```python
from build123d import *

# Parameters (mm, degrees)
LINK_PROFILE_SKETCH_R = 2.5
LINK_BAR_4MM_DEPTH    = 2


with BuildPart() as part:
    # Link Profile Sketch → Link Bar 4mm (new, symmetric)
    with BuildSketch(Plane.XY):
        with BuildLine():
            Line((-45, 5), (45, 5))
            ThreePointArc((45, 5), (50, 0), (45, -5))
            Line((45, -5), (-45, -5))
            ThreePointArc((-45, -5), (-50, 0), (-45, 5))
        make_face()
        with Locations((-45, 0)):
            Circle(LINK_PROFILE_SKETCH_R, mode=Mode.SUBTRACT)
        with Locations((45, 0)):
            Circle(LINK_PROFILE_SKETCH_R, mode=Mode.SUBTRACT)
    extrude(amount=LINK_BAR_4MM_DEPTH, both=True)


solid = part.part
```
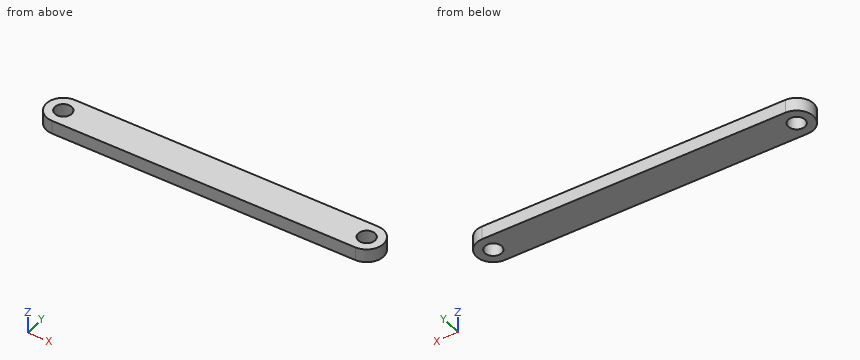
Model file for the job. Use its own axes, mm. Coordinates: 2 decimals unless noted, no trailing zeros. Order: outer loops, then holes, each group sorted by start corner. A loop starts at its lowest first (then second) coordinate and runs counter-clockwise, first axis right, second up. Notation, with made-up numbers: (52, 65.25) -> (107, 65.25) arc R26 cw to (107, 102.25) -> close; hole circle Ø6 at (5, -8.5). An arc over 180 degrees is marked (long way). Answer as a JSON object with one key per item and string values. Group by question number.
1) Drill centre lines: L1, parallel to Y at x = -45, z = 0.75; L2, parallel to X at y = 1, z = 0.4; L3, parallel to X at y = 0.5, z = -0.45. Where is each one in solid material? Low to high.
2) Cut at C-C, the plane y = 4. Write the cut outline in (x, z), then the cut area to 3 significant figures.
3) Cut at D-D, the plane y = -3.75. Write the cut outline in (x, z).
4) Cut at A-A, the plane y = 0. Write the cut outline in (x, z), then the cut area to 3 significant figures.
5) Flat gauge pins, fed straight in: pin 1 (4.5 mm diameter, centred on x = 45, y = 0, fed in from -Z); pin 2 (2 mm diameter, centred on y = -2.5, z = 1, fed in from +X). Where does each tip first touch, or does it go through?
6) Cut at B-B, the plane z = 1.4. Write the cut outline in (x, y).
Check values:
{
 "1": {"L1": "y = -5 to -2.5, 2.5 to 5", "L2": "x = -49.9 to -47.29, -42.71 to 42.71, 47.29 to 49.9", "L3": "x = -49.97 to -47.45, -42.55 to 42.55, 47.45 to 49.97"},
 "2": {"outline": "(-48, -2) -> (48, -2) -> (48, 2) -> (-48, 2) -> close", "area": "384 mm²"},
 "3": {"outline": "(-48.31, -2) -> (48.31, -2) -> (48.31, 2) -> (-48.31, 2) -> close"},
 "4": {"outline": "(-50, -2) -> (-47.5, -2) -> (-47.5, 2) -> (-50, 2) -> close; (-42.5, -2) -> (42.5, -2) -> (42.5, 2) -> (-42.5, 2) -> close; (47.5, -2) -> (50, -2) -> (50, 2) -> (47.5, 2) -> close", "area": "360 mm²"},
 "5": {"pin 1": "passes through", "pin 2": "stops at x = 49.77"},
 "6": {"outline": "(-45, -5) -> (45, -5) arc R5 ccw to (45, 5) -> (-45, 5) arc R5 ccw to start; hole circle Ø5 at (-45, 0); hole circle Ø5 at (45, 0)"}
}
